For this review, take the finished solid that the model builds, in its own axes (mm). Face numbers are marked on the shaded views. A direction names the side the tool comes from. Coordinates: 2 decimals unless noted, no trailing zeros. Loops run counter-clockwise (first coordinate to the right, second up) from the corner with the lowest first, then second, coordinate; pieces in that order, holes last. Notation, with made-up numbers: M 80.5,-4 L 116.5,-4 A21 cw 116.5,13 Z; hole C -28,21 d3. An arc over 180 degrees is marked long. Answer as a JSON object with one key per item and string values. Group by question number.
Item 1: Insertion check: pin 1 (2 mm diameter, centred on x = -3, z = 41, fed in from -Y); pin 2 (4 mm diameter, centred on x = 2.5, z = 48.5, fed in from +Y). Each pin has a flat end and moves straight along its axis. Give the tip position at first contact, or say it passes through.
Item 2: Add section B-B (y = 3.25). State the section outline as (x, z) points, then the cut area to 3 significant figures.
Item 3: Add section A-A (z = 70). State the section outline as (x, y) points, then the cut area to 3 significant figures.
Item 4: Add section C-C (x = 0). State the section outline as (y, z) points, then the cut area to 3 significant figures.
Item 5: Wall thickness on L1, parallel to X at y = 1.25, z = 66.5; L2, parallel to Z at x = -1.75, y = -3.5; L3, parallel to Z at x = 3.5, y = -2.25: over which ranges is each line inside the solid? List them lowest first. Write a range as from..to.
Item 6: Tool access review of the marked faces 1 and 2: name each direction out of +Z, -Z, +X, -X, +Y, -Y from which nothing blocks a thin tool from reaching the whole face with its end or side.
Item 7: Add section D-D (z = 18). State the section outline as (x, y) points.
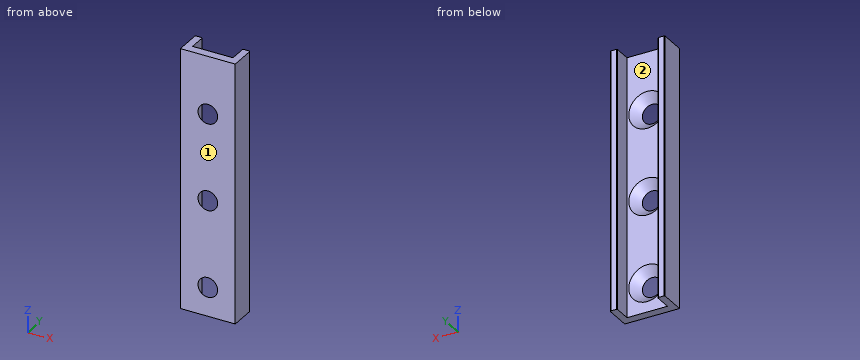
from build123d import *

# Parameters (mm, degrees)
BOSS_EXTRUDE1_DEPTH                         = 90
HOLE_SIZE_PER_HEX_SOCKET_LOBED_SEMI_2_COUNT = 2
HOLE_SIZE_PER_HEX_SOCKET_LOBED_SEMI_2_PITCH = 30
LPATTERN1_COUNT                             = 2
LPATTERN1_PITCH                             = 30
CHAMFER1_SIZE                               = 0.3


with BuildPart() as part:
    # Sketch1 → Boss-Extrude1 (new body)
    with BuildSketch(Plane.XY):
        Polygon((-7, 4.5), (-7, -1.5), (7, -1.5), (7, 4.5), (9.5, 4.5), (9.5, -4.5), (-9.5, -4.5), (-9.5, 4.5), align=None)
    extrude(amount=BOSS_EXTRUDE1_DEPTH)

    # Sketch5 → Hole size per hex socket lobed semi-countersunk screw type1 (revolve, cut)
    with BuildSketch(Plane(origin=(0, -1.5, 10), x_dir=(0, 0, 1), z_dir=(1, 0, 0))):
        Polygon((0, 0), (0, 3), (3.3, 3), (3.3, 3.1), (6.4, 0), align=None)
    hole_size_per_hex_socket_lobed_semi_coun = revolve(axis=Axis((0, 4.85, 10), (0, -1, 0)), mode=Mode.SUBTRACT)

    # Hole size per hex socket lobed semi- 2: Hole size per hex socket lobed semi-countersunk screw type1 ×2
    with Locations(*[(0, 0, i * HOLE_SIZE_PER_HEX_SOCKET_LOBED_SEMI_2_PITCH) for i in range(1, HOLE_SIZE_PER_HEX_SOCKET_LOBED_SEMI_2_COUNT)]):
        add(hole_size_per_hex_socket_lobed_semi_coun, mode=Mode.SUBTRACT)

    # LPattern1: Hole size per hex socket lobed semi-countersunk screw type1 ×2
    with Locations(*[(0, 0, i * LPATTERN1_PITCH) for i in range(1, LPATTERN1_COUNT)]):
        add(hole_size_per_hex_socket_lobed_semi_coun, mode=Mode.SUBTRACT)

    # LPattern1 copy 1 sketch → LPattern1 copy 1 (revolve, cut)
    with BuildSketch(Plane(origin=(0, -1.5, 70), x_dir=(0, 0, 1), z_dir=(1, 0, 0))):
        Polygon((0, 0), (0, 3), (3.3, 3), (3.3, 3.1), (6.4, 0), align=None)
    revolve(axis=Axis((0, 4.85, 70), (0, -1, 0)), mode=Mode.SUBTRACT)

    # Chamfer1
    chamfer1_edges = [part.edges().sort_by_distance(p)[0] for p in [
        (9.5, 4.5, 45),
        (-9.5, 4.5, 45),
        (-7, 4.5, 45),
        (7, 4.5, 45),
    ]]
    chamfer(chamfer1_edges, length=CHAMFER1_SIZE)


solid = part.part
From the geometry:
{
 "1": {"pin 1": "stops at y = -4.5", "pin 2": "stops at y = -1.5"},
 "2": {"outline": "M -9.5,0 L -7,0 L -7,90 L -9.5,90 Z; M 7,0 L 9.5,0 L 9.5,90 L 7,90 Z", "area": "450 mm²"},
 "3": {"outline": "M -9.5,-4.5 L -3.4,-4.5 L -6.4,-1.5 L -7,-1.5 L -7,4.2 L -7.3,4.5 L -9.2,4.5 L -9.5,4.2 Z; M 3.4,-4.5 L 9.5,-4.5 L 9.5,4.2 L 9.2,4.5 L 7.3,4.5 L 7,4.2 L 7,-1.5 L 6.4,-1.5 Z", "area": "57.4 mm²"},
 "4": {"outline": "M -4.5,0 L -1.5,0 L -1.5,3.6 L -4.5,6.6 Z; M -4.5,13.4 L -1.5,16.4 L -1.5,33.6 L -4.5,36.6 Z; M -4.5,43.4 L -1.5,46.4 L -1.5,63.6 L -4.5,66.6 Z; M -4.5,73.4 L -1.5,76.4 L -1.5,90 L -4.5,90 Z", "area": "182 mm²"},
 "5": {"L1": "x = -9.5..-7, 7..9.5", "L2": "z = 0..5.96, 14.04..35.96, 44.04..65.96, 74.04..90", "L3": "z = 0..5.56, 14.44..35.56, 44.44..65.56, 74.44..90"},
 "6": {"face 1": "+Z, -Z, +X, -X, -Y", "face 2": "+Z, -Z, +Y"},
 "7": {"outline": "M -9.5,-4.5 L 9.5,-4.5 L 9.5,4.2 L 9.2,4.5 L 7.3,4.5 L 7,4.2 L 7,-1.5 L -7,-1.5 L -7,4.2 L -7.3,4.5 L -9.2,4.5 L -9.5,4.2 Z"}
}
